Design review of the part built by this model. Coordinates are the model's own, in mm. Face numbers are marked on the shaded views. A direction names the side the tool comes from. Round coordinates to 2 decimals unless told otherwise and drop trailing zeros. Loops run counter-clockwise (first coordinate to the right, second up) from the corner with the lowest first, then second, coordinate; pieces in that order, holes last. Notation, with made-up numbers: (-28, 13) -> (-7, 13) arc R5 cw to (-7, 19) -> close; hole circle Ø1 at (22, 55). An arc over 180 degrees is marked (long way). Use a Markdown table: item, result. Add a question column.
from build123d import *

# Parameters (mm, degrees)
EXTRUDE_1_DEPTH             = 400
CUT_EXTRUDE_1_REACH         = 426.949
SKETCH_2_W                  = 100
SKETCH_2_H                  = 340
CUT_EXTRUDE_2_REACH         = 426.949
SKETCH_3_R                  = 13.5
SKETCH_4_R                  = 25
CUT_EXTRUDE_3_DEPTH         = 10
CUT_EXTRUDE_START           = -30
SKETCH_4_2_R                = 25
CUT_EXTRUDE_4_DEPTH         = 10
HOLE_WIZARD_13_0_13_1_D     = 13
HOLE_WIZARD_13_0_13_1_DEPTH = 70
HOLE_WIZARD_13_0_13_1_TIP   = 3.905594024


with BuildPart() as part:
    # 草图1 → 凸台-拉伸1 (new body)
    with BuildSketch(Plane.XY):
        Polygon((-107.5, 0), (107.5, 0), (107.5, 25), (65, 25), (65, 70), (85, 70), (85, 95), (-85, 95), (-85, 70), (-65, 70), (-65, 25), (-107.5, 25), align=None)
    extrude(amount=EXTRUDE_1_DEPTH)

    # 草图2 → 切除-拉伸1 (cut, up to next)
    with BuildSketch(Plane(origin=(0, 95, 0), x_dir=(1, 0, 0), z_dir=(0, 1, 0)), mode=Mode.PRIVATE) as cut_extrude_1_sk1:
        with Locations((0, -190)):
            Rectangle(SKETCH_2_W, SKETCH_2_H)
    cut_extrude_1_tool1 = extrude(cut_extrude_1_sk1.sketch, amount=-CUT_EXTRUDE_1_REACH, mode=Mode.PRIVATE) & part.part
    add(cut_extrude_1_tool1.solids().sort_by_distance((0, 95, 190))[0], mode=Mode.SUBTRACT)

    # 草图3 → 切除-拉伸2 (cut, up to next)
    with BuildSketch(Plane.XY.offset(400), mode=Mode.PRIVATE) as cut_extrude_2_sk1:
        with Locations((0, 65)):
            Circle(SKETCH_3_R)
    cut_extrude_2_tool1 = extrude(cut_extrude_2_sk1.sketch, amount=-CUT_EXTRUDE_2_REACH, mode=Mode.PRIVATE) & part.part
    add(cut_extrude_2_tool1.solids().sort_by_distance((0, 65, 400))[0], mode=Mode.SUBTRACT)

    # 草图4 → 切除-拉伸3 (cut)
    with BuildSketch(Plane.XY.offset(400)):
        with Locations((0, 65)):
            Circle(SKETCH_4_R)
    extrude(amount=-CUT_EXTRUDE_3_DEPTH, mode=Mode.SUBTRACT)

    # 草图4<2> → 切除-拉伸4 (cut)
    with BuildSketch(Plane.XY.offset(400).offset(CUT_EXTRUDE_START)):
        with Locations((0, 65)):
            Circle(SKETCH_4_2_R)
    extrude(amount=-CUT_EXTRUDE_4_DEPTH, mode=Mode.SUBTRACT)

    # Ø13.0 (13) 直径孔1
    with Locations(Plane(origin=(0, 25, 0), x_dir=(1, 0, 0), z_dir=(0, 1, 0))):
        with Locations((-92.5, -350), (92.5, -350), (-92.5, -225), (92.5, -225), (-92.5, -25), (92.5, -25)):
            Hole(HOLE_WIZARD_13_0_13_1_D / 2, depth=HOLE_WIZARD_13_0_13_1_DEPTH)
            with Locations((0, 0, -(HOLE_WIZARD_13_0_13_1_DEPTH + HOLE_WIZARD_13_0_13_1_TIP / 2))):  # 118° drill point
                Cone(0, HOLE_WIZARD_13_0_13_1_D / 2, HOLE_WIZARD_13_0_13_1_TIP, mode=Mode.SUBTRACT)


solid = part.part
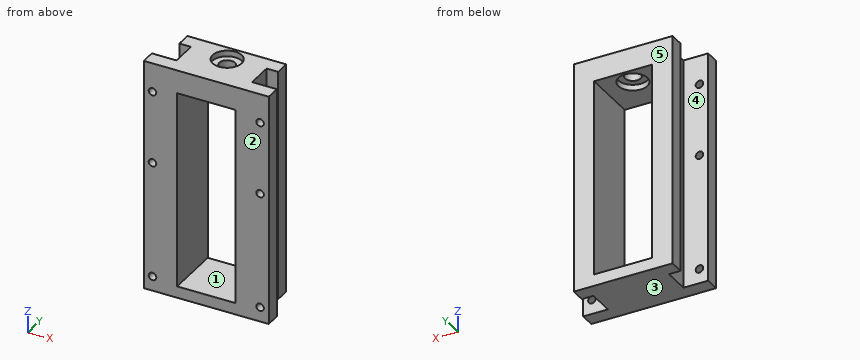
1. Consider section C-C on x = -92.5. State the section outline as (y, z) points.
2. Mouldability with a two-part tool opening along Y and no side actions: class the marked faces 3, 4 and 5 as +Y half, -Y half, draft (parallel to the pull), parting line (faces both ways), or undercut.
3. Consider section D-D on z = 47. State the section outline as (x, y) points, plus the area to 4 significant figures.
4. To check wall thickness, follow probe 1 along Z at (x, y) = (92, 8); probe 2 along X at (y, z) = (13, 350); probe 3 along Y at (x, z) = (0, 374). State the ranges of each line that lie inside material, in increasing order. Write a range as from..to.
5. For the marked faces 1 and 2, list the 3-axis set-ups (+Z, -Z, +X, -X, +Y, -Y) from which the entire face can be reached by the end or side of a thin tool; tool diameter is ignored.
6. Consider section A-A on z = 350. State the section outline as (x, y) points.
7. Consider section B-B on y = 36. State the section outline as (x, z) points.
8. Insertion check: P1, Ø5, axis at x = 45.5, z = 310.5, coming from the -Y side; P2, Ø13.5, axis at y = 38.5, z = 274, coming from the +X side; P3, Ø20, axis at y = 79, z = 145.5, coming from the -X side; P4, Ø12.5, axis at y = 87, z = 143.5, coming from the +X side. Each pin has a flat end and moves straight along its axis. Give the tip position at first contact, or say it passes through.
Verdict:
| question | item | result |
|---|---|---|
| 1 | outline | (0, 0) -> (25, 0) -> (25, 18.5) -> (0, 18.5) -> close; (0, 31.5) -> (25, 31.5) -> (25, 218.5) -> (0, 218.5) -> close; (0, 231.5) -> (25, 231.5) -> (25, 343.5) -> (0, 343.5) -> close; (0, 356.5) -> (25, 356.5) -> (25, 400) -> (0, 400) -> close |
| 2 | face 3 | draft |
| 2 | face 4 | undercut |
| 2 | face 5 | +Y half |
| 3 | outline | (-107.5, 0) -> (-50, 0) -> (-50, 95) -> (-85, 95) -> (-85, 70) -> (-65, 70) -> (-65, 25) -> (-107.5, 25) -> close; (50, 0) -> (107.5, 0) -> (107.5, 25) -> (65, 25) -> (65, 70) -> (85, 70) -> (85, 95) -> (50, 95) -> close |
| 3 | area | 5,975 mm² |
| 4 | probe 1 | z = 0..18.52, 31.48..218.52, 231.48..343.52, 356.48..400 |
| 4 | probe 2 | x = -107.5..-99, -86..-50, 50..86, 99..107.5 |
| 4 | probe 3 | y = 0..51.5, 78.5..95 |
| 5 | face 1 | +Y, -Y |
| 5 | face 2 | +Z, -Z, +X, -X, -Y |
| 6 | outline | (-107.5, 0) -> (-99, 0) -> (-99, 25) -> (-107.5, 25) -> close; (-86, 0) -> (-50, 0) -> (-50, 95) -> (-85, 95) -> (-85, 70) -> (-65, 70) -> (-65, 25) -> (-86, 25) -> close; (50, 0) -> (86, 0) -> (86, 25) -> (65, 25) -> (65, 70) -> (85, 70) -> (85, 95) -> (50, 95) -> close; (99, 0) -> (107.5, 0) -> (107.5, 25) -> (99, 25) -> close |
| 7 | outline | (-65, 0) -> (65, 0) -> (65, 400) -> (-65, 400) -> close; hole (-50, 20) -> (50, 20) -> (50, 360) -> (-50, 360) -> close |
| 8 | P1 | passes through |
| 8 | P2 | stops at x = 65 |
| 8 | P3 | stops at x = -85 |
| 8 | P4 | stops at x = 85 |
